from build123d import *

# Parameters (mm, degrees)
BOSS_EXTRUDE1_DEPTH = 20
FILLET1_R           = 50
FILLET2_R           = 20


with BuildPart() as part:
    # Sketch1 → Boss-Extrude1 (new body)
    with BuildSketch(Plane(origin=(0, 0, 0), x_dir=(1, 0, 0), z_dir=(0, 1, 0))):
        with BuildLine():
            Line((-320, 150), (-320, 30))
            ThreePointArc((-320, 30), (-343.431457505, -26.568542495), (-400, -50))
            Line((-400, -50), (-400, -150))
            Line((-400, -150), (400, -150))
            Line((400, -150), (400, -50))
            ThreePointArc((400, -50), (343.431457505, -26.568542495), (320, 30))
            Line((320, 30), (320, 150))
            Line((320, 150), (-320, 150))
        make_face()
    extrude(amount=-BOSS_EXTRUDE1_DEPTH)

    # Fillet1
    fillet1_edges = [part.edges().sort_by_distance(p)[0] for p in [
        (400, -10, 150),
        (-400, -10, 150),
    ]]
    fillet(fillet1_edges, radius=FILLET1_R)

    # Fillet2
    fillet2_edges = [part.edges().sort_by_distance(p)[0] for p in [
        (-400, -10, 50),
        (-320, -10, -150),
        (320, -10, -150),
        (400, -10, 50),
    ]]
    fillet(fillet2_edges, radius=FILLET2_R)


solid = part.part
Build history of the part. All positions in model axes, mm. A direction names the side the tool comes from. Give positions to 0.01 mm unless a question says otherwise; leave off trailing zeros. Order: outer loops, then holes, each group sorted by start corner. A loop starts at its lowest first (then second) coordinate and runs counter-clockwise, first axis right, second up. Notation, with made-up numbers: M -21.75,68.5 L 28.25,68.5 A21 ccw 28.25,74.5 Z; hole C -21,53.5 d2. An arc over 180 degrees is marked long. Put each result on its own line as item: value.
Item 1: Cut at A-A on y = -15. Write the cut outline in (x, z).
Results are:
outline: M -400,67.98 A20 ccw -384,48.38 A80 cw -320,-30 L -320,-130 A20 ccw -300,-150 L 300,-150 A20 ccw 320,-130 L 320,-30 A80 cw 384,48.38 A20 ccw 400,67.98 L 400,100 A50 ccw 350,150 L -350,150 A50 ccw -400,100 Z
Item 2: Wall check: probe 1 along X at (y, z) = (-13.25, -70); probe 2 along X at (y, z) = (-9.5, -132); probe 3 along Z at (x, y) = (350, -12). Give the ranges that are in metal, low to high.
Results are:
probe 1: -320 to 320
probe 2: -319.9 to 319.9
probe 3: 32.45 to 150
Item 3: Cut at B-B on z = -37.5. Write the cut outline in (x, y).
Results are:
outline: M -320,-20 L 320,-20 L 320,0 L -320,0 Z
Item 4: Cut at C-C on z = 9.5. Write the cut outline in (x, y).
Results are:
outline: M -330.43,-20 L 330.43,-20 L 330.43,0 L -330.43,0 Z
Item 5: Which spindle directions (+Z, -Z, +X, -X, +Y, -Y) get a long thin tool onto all of the face, cutting with end or side? Do faces 1 (the face through (-385.742, -10.14, 134.964)), 2 (the face through (-320, -10, -81)), 3 (the face through (320, -10, -79)). Say none if no direction does.
Results are:
face 1: +Z, -X, +Y, -Y
face 2: -Z, -X, +Y, -Y
face 3: -Z, +X, +Y, -Y
Item 6: Drop flat-ended pins along their axis: pin 1 Ø8 at (y, z) = (-3, 15) entering from -X; pin 2 Ø10 at (y, z) = (-6, -91) entering from +X; pin 3 Ø6 at (y, z) = (-8.5, -15.5) entering from -X. Give the stop position or say it passes through.
Results are:
pin 1: x = -336.76
pin 2: x = 320
pin 3: x = -321.94
